Design review of the part shown in the three views and the two pictorial views. Dimensions are in mm from the part's minimum x, y and z. Give positions to 0.01 mm unless a question says otherwise; leave off trailing zeros. Loops run counter-clockwise (first coordinate to the right, second up) from the corner with the lowest first, then second, coordinate; pieces in that order, holes last. Notation, with made-up numbers: (27.25, -32) - (46.25, -32) arc R13 cw to (46.25, -23) - close; hole circle Ø9 at (56.25, 62.5). An arc over 180 degrees is marked (long way). Answer in a Markdown table with one row per item.
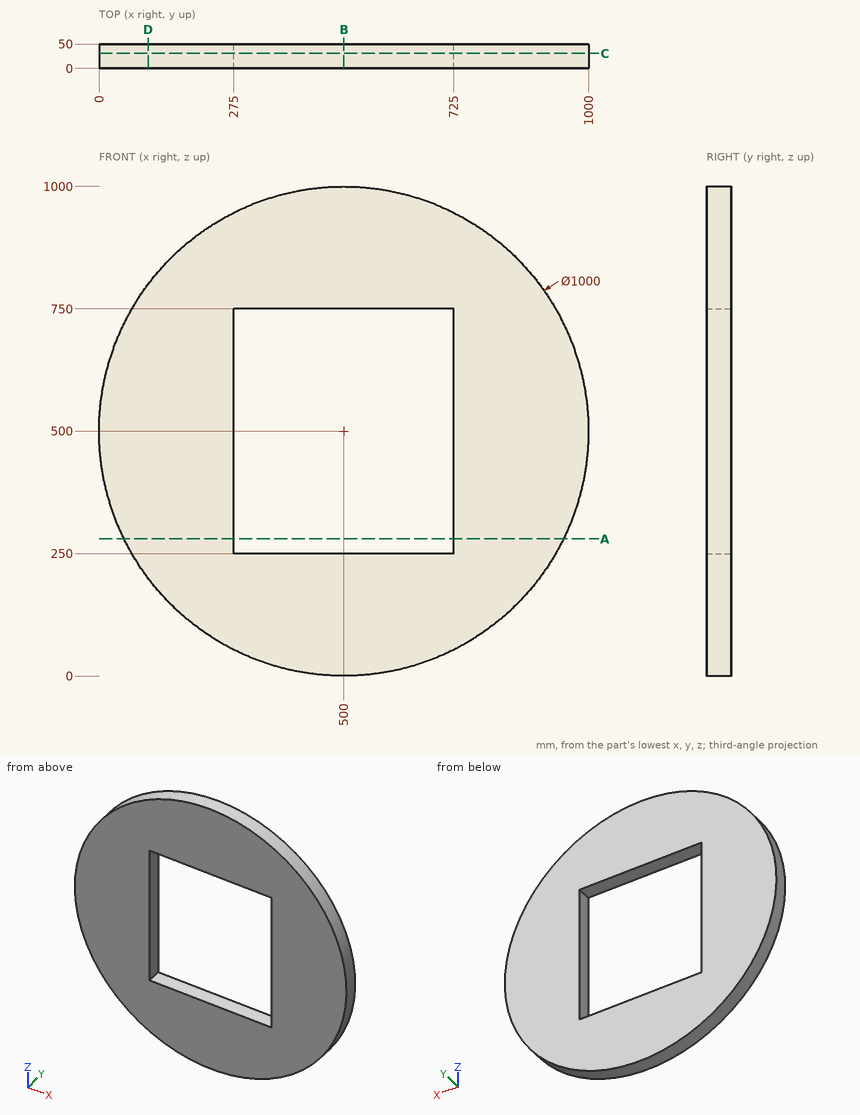
1. We need section C-C, the plane y = 31. Give the boundary of the cut face in (x, z), and give its area (3 significant figures).
Values:
| item | result |
|---|---|
| outline | circle Ø1000 at (500, 500); hole (275, 250) - (725, 250) - (725, 750) - (275, 750) - close |
| area | 560,000 mm^2 |
2. Wall thickness on line 1 (X direction, y = 33, z = 252); line 2 (X direction, y = 24, z = 490); line 3 (Z direction, x = 423.5, y = 21.5): over which ranges is each line inside the solid? List them lowest first. Write a range as [from, to].
Values:
| item | result |
|---|---|
| line 1 | x = [65.84, 275], [725, 934.16] |
| line 2 | x = [0.1, 275], [725, 999.9] |
| line 3 | z = [5.89, 250], [750, 994.11] |
3. We need section A-A, the plane z = 280. Give the boundary of the cut face in (x, y).
Values:
| item | result |
|---|---|
| outline | (51, 0) - (275, 0) - (275, 50) - (51, 50) - close; (725, 0) - (949, 0) - (949, 50) - (725, 50) - close |
4. Clearance check with flat-ended pins moving along their axes: pin 1 (4 mm diameter, centred on x = 220, y = 44.5, fed in from -Z); pin 2 (8 mm diameter, centred on y = 41, z = 116, fed in from -X); pin 3 (1.5 mm diameter, centred on x = 895, y = 18.5, fed in from -Z). State where each tip first meets the part, or that it passes through.
Values:
| item | result |
|---|---|
| pin 1 | stops at z = 84.41 |
| pin 2 | stops at x = 175.04 |
| pin 3 | stops at z = 192.48 |
5. We need section D-D, the plane x = 100.5. Give the boundary of the cut face in (y, z), and give its area (3 significant figures).
Values:
| item | result |
|---|---|
| outline | (0, 199.33) - (50, 199.33) - (50, 800.67) - (0, 800.67) - close |
| area | 30,100 mm^2 |
6. We need section B-B, the plane x = 500. Give the boundary of the cut face in (y, z).
Values:
| item | result |
|---|---|
| outline | (0, 0) - (50, 0) - (50, 250) - (0, 250) - close; (0, 750) - (50, 750) - (50, 1000) - (0, 1000) - close |
